CAD build for the part. Positions are in the model's coordinates, mm. A direction names the side the tool comes from. Give positions to 0.01 mm unless a question says otherwise; leave off trailing zeros. Loops run counter-clockwise (first coordinate to the right, second up) from the corner with the lowest first, then second, coordinate; pieces in that order, holes last. Notation, with made-up numbers: (58.25, 16) - (72.25, 16) arc R22 ccw to (72.25, 29) - close; hole circle Ø3 at (73.25, 64.5). An arc over 180 degrees is marked (long way). Return JSON: item names as keys, results as strings.
from build123d import *

# Parameters (mm, degrees)
CUT_EXTRUDE_1_DEPTH = 5


with BuildPart() as part:
    # Sketch 1 → Revolve 1 (revolve)
    with BuildSketch(Plane.XY, mode=Mode.PRIVATE) as revolve_1_sk:
        Polygon((0, 6), (-5.1, 6), (-5.1, 0), (-3, 0), (-3, -50), (0, -50), align=None)
    revolve(revolve_1_sk.sketch.rotate(Axis((0, 11.322033898, 0), (0, -1, 0)), 270), axis=Axis((0, 11.322033898, 0), (0, -1, 0)))

    # Sketch 2 → Cut-Extrude 1 (cut)
    with BuildSketch(Plane(origin=(0, 6, 0), x_dir=(1, 0, 0), z_dir=(0, 1, 0))):
        Polygon((0, 2.886751346), (-2.5, 1.443375673), (-2.5, -1.443375673), (0, -2.886751346), (2.5, -1.443375673), (2.5, 1.443375673), align=None)
    extrude(amount=-CUT_EXTRUDE_1_DEPTH, mode=Mode.SUBTRACT)


solid = part.part
1. Cut at B-B, the plane x = 1.75. Write the cut outline in (y, z), plus the area to 3 significant figures.
Values follow:
{"outline": "(-50, -2.44) - (0, -2.44) - (0, -4.79) - (6, -4.79) - (6, -1.88) - (1, -1.88) - (1, 1.88) - (6, 1.88) - (6, 4.79) - (0, 4.79) - (0, 2.44) - (-50, 2.44) - close", "area": "282 mm²"}
2. Cut at A-A, the plane z = 0. Write the cut outline in (x, y).
Values follow:
{"outline": "(-5.1, 0) - (-3, 0) - (-3, -50) - (3, -50) - (3, 0) - (5.1, 0) - (5.1, 6) - (2.5, 6) - (2.5, 1) - (-2.5, 1) - (-2.5, 6) - (-5.1, 6) - close"}
3. Drop flat-ended pins along their axis: P1, Ø1.4, axis at y = 4.5, z = 0.5, coming from the +X side; P2, Ø2, axis at x = -0.5, y = -14, coming from the -Z side; P3, Ø4, axis at y = -42, z = -0.5, coming from the +X side; P4, Ø6, axis at x = -1, y = -4, coming from the +Z side. Give the stop position or say it passes through.
Values follow:
{"P1": "stops at x = 5.1", "P2": "stops at z = -3", "P3": "stops at x = 3", "P4": "stops at z = 3"}
4. Pull direction X, two halves, no side cores. Call faces 1 (the face through (-1.532, 2.958, 4.864)), 2 (the face through (0, 1, 0)), 3 (the face through (0, -50, 0)): +X half, -X half, draft (parallel to the pull), parting line (faces both ways), or undercut.
Values follow:
{"face 1": "parting line", "face 2": "undercut", "face 3": "draft"}
5. Cut at C-C, the plane y = -46.5. Write the cut outline in (x, z), plus the area to 3 significant figures.
Values follow:
{"outline": "circle Ø6 at (0, 0)", "area": "28.3 mm²"}
6. Which spindle directions (+Z, -Z, +X, -X, +Y, -Y) get a long thin tool onto all of the face, cutting with end or side? Do faces 4 (the face through (2.5, 4, 0)), 5 (the face through (2, 6, -2)), 6 (the face through (-0.1, 0, 3.3)). Say none if no direction does.
Values follow:
{"face 4": "+Y", "face 5": "+Z, -Z, +X, -X, +Y", "face 6": "-Y"}
7. Drill centre lines: probe 1 along X at (y, z) = (-19, -0.25); probe 2 along Y at (x, z) = (-3.5, -3.5); probe 3 along Y at (x, z) = (0.5, -0.25). Where is each one in solid material? Low to high.
Values follow:
{"probe 1": "x = -2.99 to 2.99", "probe 2": "y = 0 to 6", "probe 3": "y = -50 to 1"}
